The listing builds one solid part. Answer for the finished solid, in the listing's coordinates (mm). A direction names the side the tool comes from. Coordinates: 2 decimals unless noted, no trailing zeros. Loops run counter-clockwise (first coordinate to the right, second up) from the corner with the lowest first, then second, coordinate; pieces in that order, holes last. Notation, with made-up numbers: (-20.75, 11) -> (13.25, 11) arc R18 ccw to (13.25, 26) -> close; hole circle Ø2 at (-28.75, -24.5). An arc over 180 degrees is marked (long way). Answer in a Markdown table with one row per item.
```python
from build123d import *

# Parameters (mm, degrees)
EXTRUDE_1_DEPTH = 10


with BuildPart() as part:
    # 草图1 → 凸台-拉伸1 (new body)
    with BuildSketch(Plane(origin=(0, 0, 0), x_dir=(1, 0, 0), z_dir=(0, 1, 0))):
        with BuildLine():
            Line((120, -75), (-120, -75))
            ThreePointArc((-120, -75), (-127.071067812, -72.071067812), (-130, -65))
            Line((-130, -65), (-130, 65))
            ThreePointArc((-130, 65), (-127.071067812, 72.071067812), (-120, 75))
            Line((-120, 75), (120, 75))
            ThreePointArc((120, 75), (127.071067812, 72.071067812), (130, 65))
            Line((130, 65), (130, -65))
            ThreePointArc((130, -65), (127.071067812, -72.071067812), (120, -75))
        make_face()
        with BuildLine():
            Line((-72.5, 50.5), (-97.5, 50.5))
            ThreePointArc((-97.5, 50.5), (-104.5, 57.5), (-97.5, 64.5))
            Line((-97.5, 64.5), (-72.5, 64.5))
            ThreePointArc((-72.5, 64.5), (-65.5, 57.5), (-72.5, 50.5))
        make_face(mode=Mode.SUBTRACT)
        with BuildLine():
            Line((72.5, 50.5), (97.5, 50.5))
            ThreePointArc((97.5, 50.5), (104.5, 57.5), (97.5, 64.5))
            Line((97.5, 64.5), (72.5, 64.5))
            ThreePointArc((72.5, 64.5), (65.5, 57.5), (72.5, 50.5))
        make_face(mode=Mode.SUBTRACT)
        with BuildLine():
            Line((-72.5, -50.5), (-97.5, -50.5))
            ThreePointArc((-97.5, -50.5), (-104.5, -57.5), (-97.5, -64.5))
            Line((-97.5, -64.5), (-72.5, -64.5))
            ThreePointArc((-72.5, -64.5), (-65.5, -57.5), (-72.5, -50.5))
        make_face(mode=Mode.SUBTRACT)
        with BuildLine():
            Line((72.5, -50.5), (97.5, -50.5))
            ThreePointArc((97.5, -50.5), (104.5, -57.5), (97.5, -64.5))
            Line((97.5, -64.5), (72.5, -64.5))
            ThreePointArc((72.5, -64.5), (65.5, -57.5), (72.5, -50.5))
        make_face(mode=Mode.SUBTRACT)
    extrude(amount=EXTRUDE_1_DEPTH)


solid = part.part
```
Item 1: A cutting plane is placed at B-B, the plane z = 57.5. Determine the outline of the cut face in (x, y), plus the area to 3 significant figures.
Findings below:
| item | result |
|---|---|
| outline | (-130, 0) -> (-104.5, 0) -> (-104.5, 10) -> (-130, 10) -> close; (-65.5, 0) -> (65.5, 0) -> (65.5, 10) -> (-65.5, 10) -> close; (104.5, 0) -> (130, 0) -> (130, 10) -> (104.5, 10) -> close |
| area | 1,820 mm2 |
Item 2: A cutting plane is placed at A-A, the plane x = -86. Determine the outline of the cut face in (y, z), plus the area to 3 significant figures.
Findings below:
| item | result |
|---|---|
| outline | (0, -75) -> (10, -75) -> (10, -64.5) -> (0, -64.5) -> close; (0, -50.5) -> (10, -50.5) -> (10, 50.5) -> (0, 50.5) -> close; (0, 64.5) -> (10, 64.5) -> (10, 75) -> (0, 75) -> close |
| area | 1,220 mm2 |
Item 3: A tool of negligible diameter and unlimited length cuts with its end or side. For faces 4 (the face through (2, 0, -1)), 5 (the face through (65.5, 4.93, 57.65)), from which of +Z, -Z, +X, -X, +Y, -Y can it reach the whole face along a straight path? Write none if from no direction.
Findings below:
| item | result |
|---|---|
| face 4 | +Z, -Z, +X, -X, -Y |
| face 5 | +Y, -Y |
Item 4: Find the intervals of material crossed by probe 1 along Z at (x, y) = (87.5, 2.75); probe 2 along X at (y, z) = (1, 58.5); probe 3 along X at (y, z) = (2, -63.5), in increasing order.
Findings below:
| item | result |
|---|---|
| probe 1 | z = -75 to -64.5, -50.5 to 50.5, 64.5 to 75 |
| probe 2 | x = -130 to -104.43, -65.57 to 65.57, 104.43 to 130 |
| probe 3 | x = -130 to -101.11, -68.89 to 68.89, 101.11 to 130 |
Item 5: A cutting plane is placed at C-C, the plane y = 3.5. Determine the outline of the cut face in (x, z), plus the area to 3 significant figures.
Findings below:
| item | result |
|---|---|
| outline | (-130, -65) arc R10 ccw to (-120, -75) -> (120, -75) arc R10 ccw to (130, -65) -> (130, 65) arc R10 ccw to (120, 75) -> (-120, 75) arc R10 ccw to (-130, 65) -> close; hole (-97.5, -64.5) -> (-72.5, -64.5) arc R7 ccw to (-72.5, -50.5) -> (-97.5, -50.5) arc R7 ccw to start; hole (-97.5, 50.5) -> (-72.5, 50.5) arc R7 ccw to (-72.5, 64.5) -> (-97.5, 64.5) arc R7 ccw to start; hole (72.5, -64.5) -> (97.5, -64.5) arc R7 ccw to (97.5, -50.5) -> (72.5, -50.5) arc R7 ccw to start; hole (72.5, 50.5) -> (97.5, 50.5) arc R7 ccw to (97.5, 64.5) -> (72.5, 64.5) arc R7 ccw to start |
| area | 36,900 mm2 |
Item 6: Determine the mould class of faces 1 (the face through (85, 5, -64.5)), 2 (the face through (-126.99, 4.93, 72.15)), 3 (the face through (2, 10, -1)) for opening direction Z: +Z half, -Z half, draft (parallel to the pull), parting line (faces both ways), or undercut.
Findings below:
| item | result |
|---|---|
| face 1 | undercut |
| face 2 | +Z half |
| face 3 | draft |
Item 7: A flat-ended cylindrical pin translates along its axis: pin 1 Ø1 at (x, z) = (-26, 24.5) entering from -Y. Find the tip coordinate at first contact, or state that the pin passes through.
Findings below:
| item | result |
|---|---|
| pin 1 | stops at y = 0 |
